Can you work these out from the model? Positions are in its coordinate system, mm. Face numbers are marked on the shaded views. A direction names the side the tool comes from. Give positions to 0.01 mm unless a question says otherwise; leave off trailing zeros. Loops run counter-clockwise (first coordinate to the right, second up) from the corner with the lowest first, then second, coordinate; pieces in that order, holes last. Notation, with made-up numbers: (45, 33.25) - (76, 33.25) arc R16 cw to (76, 44.25) - close; hole circle Ø4 at (-5, -1). An arc over 180 degrees is marked (long way). Answer in a Markdown table with one row per item.
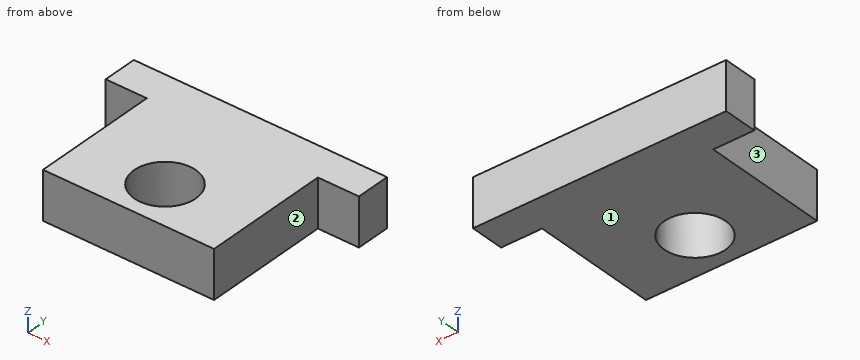
from build123d import *

# Parameters (mm, degrees)
SKETCH_1_W          = 50
SKETCH_1_H          = 47
EXTRUDE_1_DEPTH     = 7
CUT_EXTRUDE_1_REACH = 39.057
SKETCH_2_R          = 9
SKETCH_4_W          = 12
SKETCH_4_H          = 14
EXTRUDE_2_DEPTH     = 10


with BuildPart() as part:
    # 草图1 → 凸台-拉伸1 (new, symmetric)
    with BuildSketch(Plane.XY):
        Rectangle(SKETCH_1_W, SKETCH_1_H)
    extrude(amount=EXTRUDE_1_DEPTH, both=True)

    # 草图2 → 切除-拉伸1 (cut, up to next)
    with BuildSketch(Plane(origin=(0, 0, -7), x_dir=(-1, 0, 0), z_dir=(0, 0, -1)), mode=Mode.PRIVATE) as cut_extrude_1_sk1:
        with Locations((0, -10.5)):
            Circle(SKETCH_2_R)
    cut_extrude_1_tool1 = extrude(cut_extrude_1_sk1.sketch, amount=-CUT_EXTRUDE_1_REACH, mode=Mode.PRIVATE) & part.part
    add(cut_extrude_1_tool1.solids().sort_by_distance((0, -10.5, -7))[0], mode=Mode.SUBTRACT)

    # 草图4 → 凸台-拉伸2 (add)
    with BuildSketch(Plane(origin=(0, 23.5, 0), x_dir=(1, 0, 0), z_dir=(0, 1, 0))):
        with Locations((31, 0)):
            Rectangle(SKETCH_4_W, SKETCH_4_H)
        with Locations((-31, 0)):
            Rectangle(SKETCH_4_W, SKETCH_4_H)
    extrude(amount=-EXTRUDE_2_DEPTH)


solid = part.part
Q1. Imagine slicing it at B-B, the plane y = -10.5. Write out the boundary of the cut face in (x, z).
Checked values:
| item | result |
|---|---|
| outline | (-25, -7) - (-9, -7) - (-9, 7) - (-25, 7) - close; (9, -7) - (25, -7) - (25, 7) - (9, 7) - close |
Q2. Imagine slicing it at C-C, the plane z = 4.5. Write out the boundary of the cut face in (x, y).
Checked values:
| item | result |
|---|---|
| outline | (-37, 13.5) - (-25, 13.5) - (-25, -23.5) - (25, -23.5) - (25, 13.5) - (37, 13.5) - (37, 23.5) - (-37, 23.5) - close; hole circle Ø18 at (0, -10.5) |
Q3. On a 3-axis mill with a long thin cutter (end or side, diameter ignored), from which of +Z, -Z, +X, -X, +Y, -Y can I reach the whole of each face in a straight line? I mean the marked faces 1, 2 and 3. Say none if no direction works.
Checked values:
| item | result |
|---|---|
| face 1 | -Z, +X, -X, +Y, -Y |
| face 2 | +Z, -Z, +X, -Y |
| face 3 | +Z, -Z, -X, -Y |
Q4. Imagine slicing it at D-D, the plane y = 6.5. Write out the boundary of the cut face in (x, z), and give its area (3 significant figures).
Checked values:
| item | result |
|---|---|
| outline | (-25, -7) - (25, -7) - (25, 7) - (-25, 7) - close |
| area | 700 mm² |
Q5. If I drill on line 1 (Y direction, x = 0, z = 3.5); line 2 (X direction, y = 5.5, z = -1.5); line 3 (Y direction, x = -3.5, z = 2.5), over which ranges is the centre line in solid material (lowest first)? Write a range as [from, to].
Checked values:
| item | result |
|---|---|
| line 1 | y = [-23.5, -19.5], [-1.5, 23.5] |
| line 2 | x = [-25, 25] |
| line 3 | y = [-23.5, -18.79], [-2.21, 23.5] |
Q6. Imagine slicing it at A-A, the plane x = 0. Write out the boundary of the cut face in (y, z), and give its area (3 significant figures).
Checked values:
| item | result |
|---|---|
| outline | (-23.5, -7) - (-19.5, -7) - (-19.5, 7) - (-23.5, 7) - close; (-1.5, -7) - (23.5, -7) - (23.5, 7) - (-1.5, 7) - close |
| area | 406 mm² |
Q7. For pin 1 (1 mm diameter, centred on y = 3, z = 4.5, fed in from +X); pin 2 (4 mm diameter, centred on y = -3.5, z = 5, fed in from -X), each with a flat end and sliding along its axis, tell me the tip position at first contact or that it passes through.
Checked values:
| item | result |
|---|---|
| pin 1 | stops at x = 25 |
| pin 2 | stops at x = -25 |
